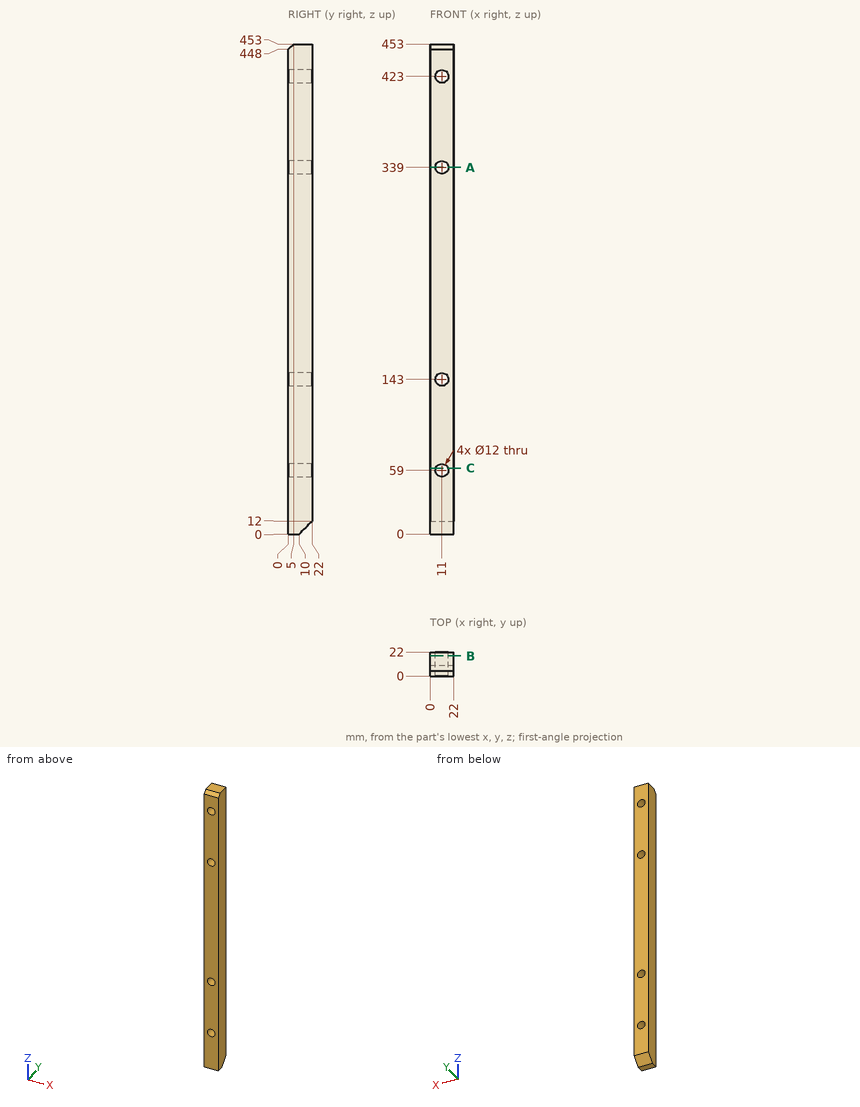
Can you work these out from the drawing? Everything is in mm from the part's minimum corner. Give positions to 0.01 mm unless a question says otherwise; leave off trailing zeros. Order: outer loops, then holes, each group sorted by start corner. A loop starts at its lowest first (then second) coordinate and runs counter-clockwise, first axis right, second up. Notation, with made-up numbers: (40.5, 46) -> (66.5, 46) arc R14 cw to (66.5, 63) -> close; hole circle Ø2 at (53, -31). An arc over 180 degrees is marked (long way). Return JSON: item names as keys, results as strings.
1. Imagine slicing it at A-A on z = 339. List the corners of the cut face in (x, y) for me.
Answer list:
{"outline": "(0, 0) -> (5, 0) -> (5, 22) -> (0, 22) -> close; (17, 0) -> (22, 0) -> (22, 22) -> (17, 22) -> close"}
2. I need wall thicknesses on line 1 (X direction, y = 8, z = 143); line 2 (Z direction, x = 6.25, y = 2.75); line 3 (Z direction, x = 7.75, y = 4.5). Which ranges of each line are inside material? Lowest first, please. Write a range as from..to.
Answer list:
{"line 1": "x = 0..5, 17..22", "line 2": "z = 0..55.33, 62.67..139.33, 146.67..335.33, 342.67..419.33, 426.67..450.75", "line 3": "z = 0..53.96, 64.04..137.96, 148.04..333.96, 344.04..417.96, 428.04..452.5"}
3. Imagine slicing it at C-C on z = 61. List the corners of the cut face in (x, y) for me, then the cut area to 3 significant figures.
Answer list:
{"outline": "(0, 0) -> (5.34, 0) -> (5.34, 22) -> (0, 22) -> close; (16.66, 0) -> (22, 0) -> (22, 22) -> (16.66, 22) -> close", "area": "235 mm2"}
4. Imagine slicing it at B-B on y = 18.5. List the corners of the cut face in (x, z) for me.
Answer list:
{"outline": "(0, 8.5) -> (22, 8.5) -> (22, 453) -> (0, 453) -> close; hole circle Ø12 at (11, 59); hole circle Ø12 at (11, 143); hole circle Ø12 at (11, 339); hole circle Ø12 at (11, 423)"}
